Source: CAD feature listing. Evaluate the final solid. Frame: model axes, mm. A direction names the side the tool comes from. Coordinates: 2 decimals unless noted, no trailing zeros. Write each loop counter-clockwise with the first axis right and the second up, starting at its lowest first coordinate (ties: lowest second). Pieces come first, ordered by that corner, then holes. Notation, with made-up numbers: M -27.5,80.5 L 29.5,80.5 A24 cw 29.5,90.5 Z; hole C -4,-36.75 d6. An arc over 180 degrees is marked long. One line per item, written item: value. Start each with the question number.
Item 1: Mould query, pull axis Y, two halves, no side actions, for faces 3 (the flat face through (0, 99, 6)), 4 (the flat face through (37, 0, 6)), 5 (the flat face through (42.97, 189.32, 6.4)). Classes: released by +Y, released by -Y, zero draft, split by the parting line, or undercut.
Item 2: Cut plane B-B, the plane x = 56. Output: boundary loops of the cut face in (y, z).
Item 3: Cut plane A-A, the plane z = 208. Output: boundary loops of the cut face in (x, y).
Item 4: Set-up query: faces 1 (the flat face through (6.6, 99.5, 457.2)), 2 (the flat face through (7, 101, 6)). Return all of +Z, -Z, +X, -X, +Y, -Y with unobstructed straight access to the full face (end or side cutting, diameter ignored); none if empty.
Item 5: Ray query, L1, parallel to Y at x = 67.5, z = 262.5; L2, parallel to Y at x = 19.5, z = 301; L3, parallel to X at y = 144, z = 302. Return the intervals inside material, ascending. Write a range as from..to.
Item 6: Pin query (flat end, axial travel): P1, Ø12, axis at y = 166.5, z = 168, coming from the +X side. Return the tip coordinate at first contact, or that it passes through.
Item 7: Cut plane C-C, the plane y = 36. Output: boundary loops of the cut face in (x, z).
```python
from build123d import *

# Parameters (mm, degrees)
BOSS_EXTRUDE1_DEPTH = 457.2


with BuildPart() as part:
    # Sketch1 → Boss-Extrude1 (new, symmetric)
    with BuildSketch(Plane(origin=(28.211262136, 0, 0), x_dir=(-1, 0, 0), z_dir=(0, 0, 1))):
        with BuildLine():
            Line((28.211262136, 0), (28.211262136, -200))
            Line((28.211262136, -200), (-44.788737864, -200))
            Line((-44.788737864, -200), (-44.788737864, -196.033179359))
            ThreePointArc((-44.788737864, -196.033179359), (-43.272315441, -192.240936001), (-39.559243433, -190.539835501))
            Line((-39.559243433, -190.539835501), (10.752273273, -188.062374452))
            ThreePointArc((10.752273273, -188.062374452), (18.17841729, -184.660173452), (21.211262136, -177.075686736))
            Line((21.211262136, -177.075686736), (21.211262136, -22.924313264))
            ThreePointArc((21.211262136, -22.924313264), (18.17841729, -15.339826548), (10.752273273, -11.937625548))
            Line((10.752273273, -11.937625548), (-39.559243433, -9.460164499))
            ThreePointArc((-39.559243433, -9.460164499), (-43.272315441, -7.759063999), (-44.788737864, -3.966820641))
            Line((-44.788737864, -3.966820641), (-44.788737864, 0))
            Line((-44.788737864, 0), (28.211262136, 0))
        make_face()
    extrude(amount=BOSS_EXTRUDE1_DEPTH, both=True)


solid = part.part
```
From the geometry:
1. face 3: zero draft
1. face 4: released by -Y
1. face 5: undercut
2. outline: M 0,-457.2 L 10.04,-457.2 L 10.04,457.2 L 0,457.2 Z; M 189.96,-457.2 L 200,-457.2 L 200,457.2 L 189.96,457.2 Z
3. outline: M 0,0 L 73,0 L 73,3.97 A5.5 ccw 67.77,9.46 L 17.46,11.94 A11 cw 7,22.92 L 7,177.08 A11 cw 17.46,188.06 L 67.77,190.54 A5.5 ccw 73,196.03 L 73,200 L 0,200 Z
4. face 1: +Z, +X, -X, +Y, -Y
4. face 2: +Z, -Z, +X
5. L1: y = 0..9.47, 190.53..200
5. L2: y = 0..11.84, 188.16..200
5. L3: x = 0..7
6. P1: stops at x = 7
7. outline: M 0,-457.2 L 7,-457.2 L 7,457.2 L 0,457.2 Z
